Input: dimensioned drawing with shaded views. Units: mm. Origin: part minimum x, y, z. A direction names the side the tool comes from. Round coordinates to 2 decimals unless told otherwise and drop trailing zeros. Loops run counter-clockwise (first coordinate to the right, second up) from the corner with the lowest first, then second, coordinate; pieces in that order, holes last. Notation, with made-up numbers: (6, 32) - (46, 32) arc R28 ccw to (46, 68) - close; hole circle Ø7 at (-40, 66.5). An arc over 180 degrees is marked (long way). Answer as CSV lines item,"result".
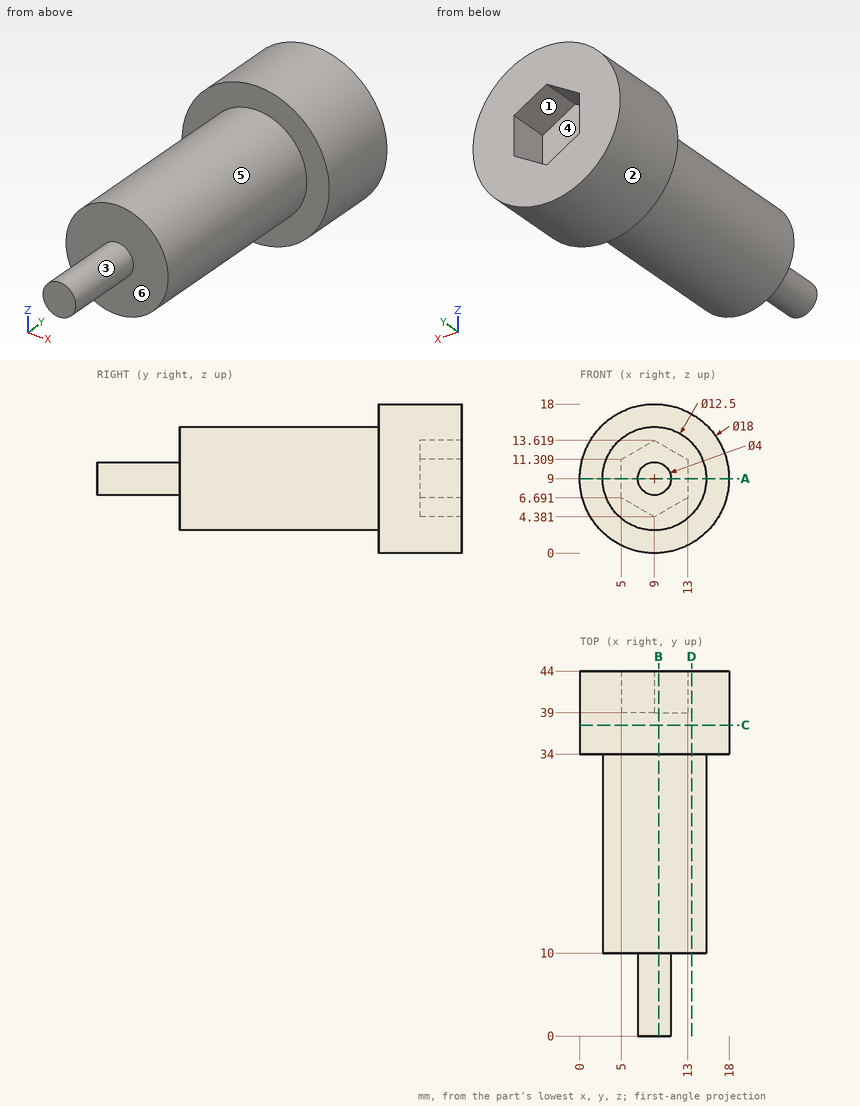
(1) Material intervals for line 1 along Y through (x, z) = (17, 12.5); line 2 along Y through (x, z) = (14, 10); line 3 along Z through (x, y) = (9.25, 31) (1 decimal), sorted ascending.
Findings below:
line 1,"34 to 44"
line 2,"10 to 44"
line 3,"2.8 to 15.2"
(2) Access query for the marked faces 1, 2 and 3. Directions: +Z, -Z, +X, -X, +Y, -Y. A direction counts if a zero-diameter tool reaches every point of the face in a straight line with its end or side. Return the directions, or none.
Findings below:
face 1,"+Y"
face 2,"+Y, -Y"
face 3,"-Y"
(3) Section C-C (y = 37.5). Output: boundary loops of the cut face in (x, z).
Findings below:
outline,"circle Ø18 at (9, 9)"
(4) Section D-D (x = 13.5). Output: boundary loops of the cut face in (y, z) (1 decimal).
Findings below:
outline,"(10, 4.7) - (34, 4.7) - (34, 1.2) - (44, 1.2) - (44, 16.8) - (34, 16.8) - (34, 13.3) - (10, 13.3) - close"
(5) Draft query along X for the marked faces 4, 5 and 6. Return one class per face: pulls with the +X half, pulls with the -X half, needs draft (parallel to the pull), parting line crosses it, or undercut.
Findings below:
face 4,"undercut"
face 5,"parting line crosses it"
face 6,"needs draft"
(6) Pin query (flat end, axial travel): P1, Ø6, axis at y = 21.5, z = 7, coming from the +X side; P2, Ø6, axis at y = 23, z = 8.5, coming from the -X side; P3, Ø4, axis at x = 10, z = 8, coming from the +Y side. Return the tip coordinate at first contact, or that it passes through.
Findings below:
P1,"x = 15.25"
P2,"x = 2.75"
P3,"y = 39"
(7) Section A-A (z = 9). Output: boundary loops of the cut face in (x, y), and give its area (3 significant figures).
Findings below:
outline,"(0, 34) - (2.75, 34) - (2.75, 10) - (7, 10) - (7, 0) - (11, 0) - (11, 10) - (15.25, 10) - (15.25, 34) - (18, 34) - (18, 44) - (13, 44) - (13, 39) - (5, 39) - (5, 44) - (0, 44) - close"
area,"480 mm2"
(8) Section B-B (x = 9.5). Output: boundary loops of the cut face in (y, z).
Findings below:
outline,"(0, 7.06) - (10, 7.06) - (10, 2.77) - (34, 2.77) - (34, 0.01) - (44, 0.01) - (44, 4.67) - (39, 4.67) - (39, 13.33) - (44, 13.33) - (44, 17.99) - (34, 17.99) - (34, 15.23) - (10, 15.23) - (10, 10.94) - (0, 10.94) - close"
